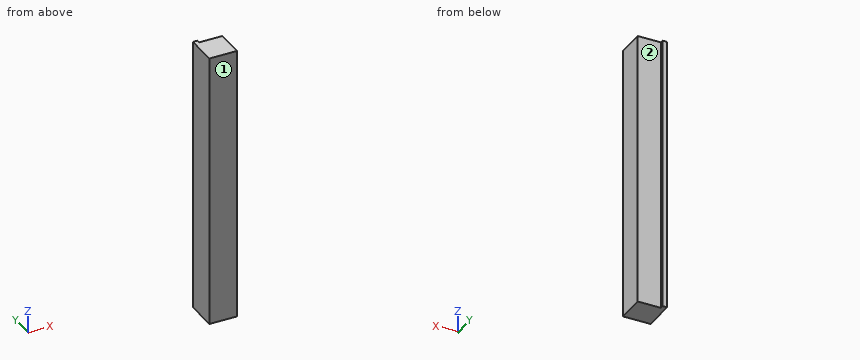
from build123d import *

# Parameters (mm, degrees)
EXTRUDE_1_DEPTH = 250


with BuildPart() as part:
    # 草图1 → 凸台-拉伸1 (new body)
    with BuildSketch(Plane.XY):
        Polygon((-10, -12.5), (-14, -12.5), (-14, -41), (11, -41), (11, -15.5), (-10, -15.5), align=None)
    extrude(amount=-EXTRUDE_1_DEPTH)


solid = part.part
Geometry: final body of the model. Coordinates: model frame, mm. Face numbers are marked on the shaded views. A direction names the side the tool comes from. Round coordinates to 2 decimals unless told otherwise and drop trailing zeros. Order: outer loops, then holes, each group sorted by start corner. A loop starts at its lowest first (then second) coordinate and runs counter-clockwise, first axis right, second up. Notation, with made-up numbers: (19, -19.5) -> (56, -19.5) arc R26 cw to (56, 7.5) -> close; hole circle Ø9 at (-17, -32). An arc over 180 degrees is marked (long way). Put each result on its own line as item: value. Start each with the question number.
Q1. Reachability of the marked faces 1 and 2 from +Z, -Z, +X, -X, +Y, -Y: full face, straight path, thin tool, end or side. Return the list, or none.
Q2. Section A-A on z = -170.5. Return the cut outline in (x, y), and give its area (4 significant figures).
Q3. Line query: probe 1 along Y at (x, z) = (8.5, -223.5); probe 2 along X at (y, z) = (-15, -43.5). Output: solid intervals per line, ascending.
Q4. First-contact query: pin 1 (2 mm diameter, centred on x = -6.5, z = -42.5, fed in from +Y). Flat tip, straight axial feed; report the tip coordinate or a pass-through.
Q5. Section B-B on x = 5. Return the cut outline in (y, z), and give its area (4 significant figures).
Ans:
1. face 1: +Z, -Z, +X, -X, -Y
1. face 2: +Z, -Z, +X, +Y
2. outline: (-14, -41) -> (11, -41) -> (11, -15.5) -> (-10, -15.5) -> (-10, -12.5) -> (-14, -12.5) -> close
2. area: 649.5 mm2
3. probe 1: y = -41 to -15.5
3. probe 2: x = -14 to -10
4. pin 1: stops at y = -15.5
5. outline: (-41, -250) -> (-15.5, -250) -> (-15.5, 0) -> (-41, 0) -> close
5. area: 6,375 mm2
